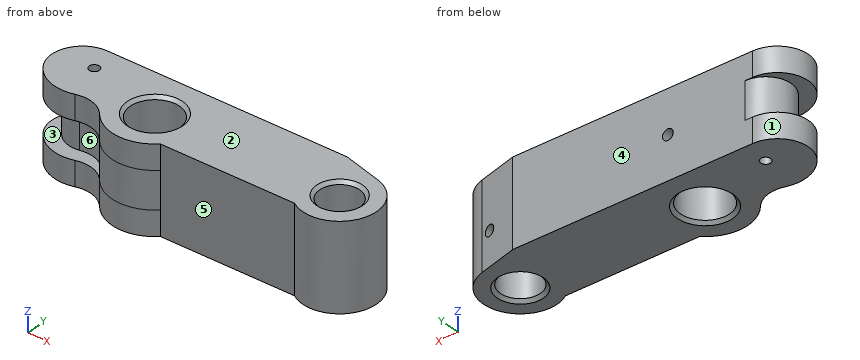
from build123d import *

# Parameters (mm, degrees)
SKETCH1_R               = 8
SKETCH1_R_2             = 6.5
SKETCH1_R_3             = 1.5
BOSS_EXTRUDE1_DEPTH     = 6
SKETCH2_R               = 6.5
SKETCH2_R_2             = 8
BOSS_EXTRUDE2_DEPTH     = 8
CUT_EXTRUDE1_REACH      = 80.873
CUT_EXTRUDE1_END_RADIUS = 8
SKETCH4_R               = 1.75
CUT_EXTRUDE2_REACH      = 80.873
CUT_EXTRUDE2_END_RADIUS = 6.5
SKETCH5_R               = 1.75
CHAMFER1_SIZE           = 1


with BuildPart() as part:
    # Sketch1 → Boss-Extrude1 (new, symmetric)
    with BuildSketch(Plane.XY):
        with BuildLine():
            Line((9.797958971, -10), (53.366750419, -10))
            ThreePointArc((53.366750419, -10), (70.93867824, -4.934097522), (63.105828541, 11.591109915))
            Line((63.105828541, 11.591109915), (50.382575949, 15.000295173))
            Line((50.382575949, 15.000295173), (-25.114071484, 15.000295173))
            ThreePointArc((-25.114071484, 15.000295173), (-33.338477244, 5.852602019), (-23.370562784, -1.355852842))
            ThreePointArc((-23.370562784, -1.355852842), (-17.0207139, -2.075403858), (-12.40317439, -6.493170646))
            ThreePointArc((-12.40317439, -6.493170646), (-2.184319087, -13.828548374), (9.797958971, -10))
        make_face()
        Circle(SKETCH1_R, mode=Mode.SUBTRACT)
        with Locations((60, 0)):
            Circle(SKETCH1_R_2, mode=Mode.SUBTRACT)
        with Locations((-25.114071484, 6.729295173)):
            Circle(SKETCH1_R_3, mode=Mode.SUBTRACT)
    extrude(amount=BOSS_EXTRUDE1_DEPTH, both=True)

    # Sketch2 → Boss-Extrude2 (add)
    with BuildSketch(Plane.XY.offset(6)):
        with BuildLine():
            Line((50.382575949, 15.000295173), (-27.565715626, 15.000295173))
            ThreePointArc((-27.565715626, 15.000295173), (-36.443590747, 9.602830706), (-35.737862766, -0.763038161))
            ThreePointArc((-35.737862766, -0.763038161), (-29.354690281, -5.559608449), (-21.371826468, -5.720427806))
            ThreePointArc((-21.371826468, -5.720427806), (-15.596757504, -5.725786931), (-10.787686266, -8.923330377))
            ThreePointArc((-10.787686266, -8.923330377), (-0.731228007, -13.98089073), (9.797958971, -10))
            Line((9.797958971, -10), (53.366750419, -10))
            ThreePointArc((53.366750419, -10), (70.93867824, -4.934097522), (63.105828541, 11.591109915))
            Line((63.105828541, 11.591109915), (50.382575949, 15.000295173))
        make_face()
        with Locations((60, 0)):
            Circle(SKETCH2_R, mode=Mode.SUBTRACT)
        Circle(SKETCH2_R_2, mode=Mode.SUBTRACT)
    boss_extrude2 = extrude(amount=BOSS_EXTRUDE2_DEPTH)

    # Mirror1: Boss-Extrude2 across plane
    add(boss_extrude2.mirror(Plane.XY))

    # Sketch3 → M4 Tapped Hole1 (revolve, cut)
    with BuildSketch(Plane(origin=(-25.114071484, 6.729295173, 14), x_dir=(0, -1, 0), z_dir=(1, 0, 0))):
        Polygon((0, 0), (0, 8.991420021), (1.65, 8), (1.65, 0), align=None)
    m4_tapped_hole1 = revolve(axis=Axis((-25.114071484, 6.729295173, 20.35), (0, 0, -1)), mode=Mode.SUBTRACT)

    # Mirror2: M4 Tapped Hole1 across plane
    add(m4_tapped_hole1.mirror(Plane.XY), mode=Mode.SUBTRACT)

    # Cut-Extrude1: up to this cylinder (the profile starts outside it)
    cut_extrude1_end = Plane(origin=(0, 0, 0), z_dir=(0, 0, -1)) * Cylinder(CUT_EXTRUDE1_END_RADIUS, 178.746, mode=Mode.PRIVATE)
    # Sketch4 → Cut-Extrude1 (cut, up to the surface)
    with BuildSketch(Plane(origin=(0, 15.000295173, 0), x_dir=(1, 0, 0), z_dir=(0, 1, 0)), mode=Mode.PRIVATE) as cut_extrude1_sk1:
        with Locations(Location((0, 0, 0), (0, 0, 180))):
            Circle(SKETCH4_R)
    cut_extrude1_tool1 = extrude(cut_extrude1_sk1.sketch, amount=-CUT_EXTRUDE1_REACH, mode=Mode.PRIVATE) - cut_extrude1_end
    add(cut_extrude1_tool1.solids().sort_by_distance((0, 15.000295, 0))[0], mode=Mode.SUBTRACT)

    # Cut-Extrude2: up to this cylinder (the profile starts outside it)
    cut_extrude2_end = Plane(origin=(60, 0, -3), z_dir=(0, 0, -1)) * Cylinder(CUT_EXTRUDE2_END_RADIUS, 175.746, mode=Mode.PRIVATE)
    # Sketch5 → Cut-Extrude2 (cut, up to the surface)
    with BuildSketch(Plane(origin=(0, 15.000295173, 0), x_dir=(1, 0, 0), z_dir=(0, 1, 0)), mode=Mode.PRIVATE) as cut_extrude2_sk1:
        with Locations(Location((60, 3, 0), (0, 0, 180))):
            Circle(SKETCH5_R)
    cut_extrude2_tool1 = extrude(cut_extrude2_sk1.sketch, amount=-CUT_EXTRUDE2_REACH, mode=Mode.PRIVATE) - cut_extrude2_end
    add(cut_extrude2_tool1.solids().sort_by_distance((60, 15.000295, -3))[0], mode=Mode.SUBTRACT)

    # Chamfer1
    chamfer1_edges = [part.edges().sort_by_distance(p)[0] for p in [
        (53.5, 0, 14),
        (-8, 0, 14),
        (-8, 0, -14),
        (53.5, 0, -14),
    ]]
    chamfer(chamfer1_edges, length=CHAMFER1_SIZE)


solid = part.part
The listing builds one solid part. Answer for the finished solid, in the listing's coordinates (mm). Face numbers are marked on the shaded views. A direction names the side the tool comes from. Round coordinates to 2 decimals unless told otherwise and drop trailing zeros. Order: outer loops, then holes, each group sorted by start corner. A loop starts at its lowest first (then second) coordinate and runs counter-clockwise, first axis right, second up. Notation, with made-up numbers: M -11.75,-31 L 14.25,-31 A26 cw 14.25,2 Z; hole C -24.75,17 d5. An arc over 180 degrees is marked long. Answer in a Markdown table with one row per item. Add a question column.
1) The part is cut by section B-B on z = 0. Determine the outline of the cut face in (x, y), plus the area to 3 significant figures.
2) Consider line 1 along Y through (x, z) = (0, 7); line 2 along X through (y, z) = (-0.75, 7.25); line 3 along X through (y, z) = (-4.5, 6.5). Determine where each line is inside the solid, lowest interval first. Write a range as from..to.
3) Flat-ended cylindrical pins translate along their axes: pin 1 Ø13 at (x, y) = (0, 0) entering from +Z; pin 2 Ø4.5 at (x, z) = (60, -3) entering from -Y; pin 3 Ø2 at (x, z) = (25, -7.5) entering from -Y; pin 4 Ø2 at (y, z) = (-1.5, 10.5) entering from +X. Find the tip coordinate at first contact, or state that the pin passes through.
4) Determine the mould class of the marked faces 1, 2 and 3 for opening direction Z: pulls with the +Z half, pulls with the -Z half, needs draft (parallel to the pull), parting line crosses it, or undercut.
5) The part is cut by section D-D on x = 23. Determine the outline of the cut face in (y, z).
6) The part is cut by section A-A on x = 0. Determine the outline of the cut face in (y, z).
7) The part is cut by section C-C on z = -7. Determine the outline of the cut face in (x, y), plus the area to 3 significant figures.
8) Which of the six approach directions +Z, -Z, +X, -X, +Y, -Y give full straight-line access (tool end or side, diameter ignored) to the marked faces 4, 5 and 6?
Findings below:
| question | item | result |
|---|---|---|
| 1 | outline | M -25.11,15 A8.27 ccw long -23.37,-1.36 A10 cw -12.4,-6.49 A14 ccw 9.8,-10 L 53.37,-10 A12 ccw long 63.11,11.59 L 50.38,15 L 1.75,15 L 1.75,7.81 A8 cw long -1.75,7.81 L -1.75,15 Z; hole C -25.11,6.73 d3; hole C 60,0 d13 |
| 1 | area | 2,040 mm² |
| 2 | line 1 | y = -14..-8, 8..15 |
| 2 | line 2 | x = -35.75..-7.96, 7.96..53.54, 66.46..71.98 |
| 2 | line 3 | x = -31.66..-6.61, 6.61..55.31, 64.69..71.12 |
| 3 | pin 1 | passes through |
| 3 | pin 2 | stops at y = -12 |
| 3 | pin 3 | stops at y = -10 |
| 3 | pin 4 | stops at x = 71.99 |
| 4 | face 1 | needs draft |
| 4 | face 2 | pulls with the +Z half |
| 4 | face 3 | undercut |
| 5 | outline | M -10,-14 L 15,-14 L 15,14 L -10,14 Z |
| 6 | outline | M -14,-14 L -9,-14 L -8,-13 L -8,13 L -9,14 L -14,14 Z; M 8,-13 L 9,-14 L 15,-14 L 15,-1.75 L 8,-1.75 Z; M 8,1.75 L 15,1.75 L 15,14 L 9,14 L 8,13 Z |
| 7 | outline | M -35.74,-0.76 A13 ccw -21.37,-5.72 A10 cw -10.79,-8.92 A14 ccw 9.8,-10 L 53.37,-10 A12 ccw long 63.11,11.59 L 50.38,15 L -27.57,15 A10 ccw Z; hole C -25.11,6.73 d3.3; hole C 0,0 d16; hole C 60,0 d13 |
| 7 | area | 2,220 mm² |
| 8 | face 4 | +Z, -Z, +X, -X, +Y |
| 8 | face 5 | +Z, -Z, -Y |
| 8 | face 6 | -Y |
